Job drawing, mm, ordinate dimensions from the low corner. One solid piece. Give positions to 0.01 mm unless a question says otherwise; leave off trailing zeros. Loops run counter-clockwise (first coordinate to the right, second up) from the corner with the lowest first, then second, coordinate; pieces in that order, holes last. Notation, with made-up numbers: (-15, 34.25) - (8, 34.25) arc R10 ccw to (8, 48.25) - close; hole circle Ø2 at (-18, 56). An arc over 180 degrees is marked (long way). Use a Markdown table: item, result.
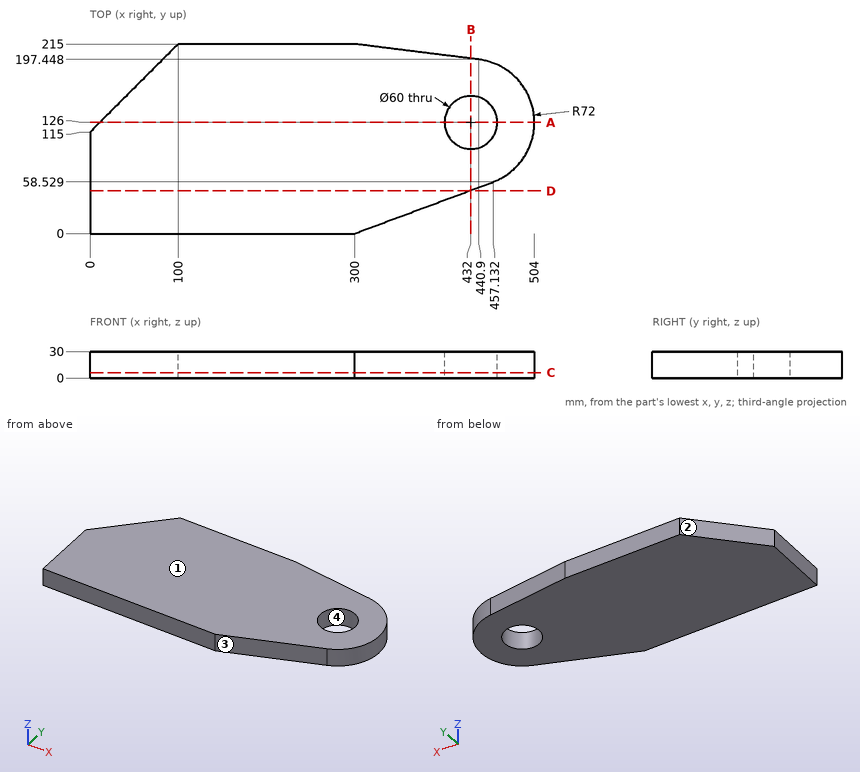
(1) Mould opens along X. For the marked faces 1, 2, 3 and 4 say: pulls with the +X half, pulls with the -X half, needs draft (parallel to the pull), parting line crosses it, or undercut.
Computed:
| item | result |
|---|---|
| face 1 | needs draft |
| face 2 | pulls with the -X half |
| face 3 | pulls with the +X half |
| face 4 | undercut |
(2) Slice it at C-C, the plane z = 6. Write the cut outline in (x, y), plus the area to 3 significant figures.
Computed:
| item | result |
|---|---|
| outline | (0, 0) - (300, 0) - (457.13, 58.53) arc R72 ccw to (440.9, 197.45) - (300, 215) - (100, 215) - (0, 115) - close; hole circle Ø60 at (432, 126) |
| area | 88,900 mm² |
(3) Pin check, flat tips, straight feed: P1, Ø8, axis at y = 172, z = 18, coming from the -X side; P2, Ø5, axis at y = 107, z = 4.5, coming from the +X side. Stop position of each tip, or through.
Computed:
| item | result |
|---|---|
| P1 | x = 53 |
| P2 | x = 502.08 |
(4) Slice it at B-B, the plane x = 432. Write the cut outline in (y, z).
Computed:
| item | result |
|---|---|
| outline | (49.17, 0) - (96, 0) - (96, 30) - (49.17, 30) - close; (156, 0) - (198.56, 0) - (198.56, 30) - (156, 30) - close |
(5) Slice it at A-A, the plane y = 126. Write the cut outline in (x, z), plus the area to 3 significant figures.
Computed:
| item | result |
|---|---|
| outline | (11, 0) - (402, 0) - (402, 30) - (11, 30) - close; (462, 0) - (504, 0) - (504, 30) - (462, 30) - close |
| area | 13,000 mm² |
(6) Drill centre lines: probe 1 along Y at (x, z) = (432, 23.25); probe 2 along X at (y, z) = (151, 14) (1 decimal); probe 3 along Y at (x, z) = (330.5, 23). Where is each one in solid material? Low to high. Write a range as [from, to].
Computed:
| item | result |
|---|---|
| probe 1 | [49.17, 96], [156, 198.56] |
| probe 2 | [36, 415.4], [448.6, 499.5] |
| probe 3 | [11.36, 211.2] |
(7) Slice it at D-D, the plane y = 48.5. Write the cut outline in (x, z).
Computed:
| item | result |
|---|---|
| outline | (0, 0) - (430.21, 0) - (430.21, 30) - (0, 30) - close |
